```python
from build123d import *

# Parameters (mm, degrees)
SKETCH_1_W                   = 45
SKETCH_1_H                   = 15
SKETCH_1_R                   = 1.55
EXTRUDE_1_DEPTH              = 2
FILLET_1_R                   = 3
HOLE_WIZARD_M3_1_D           = 3.2
HOLE_WIZARD_M3_1_DEPTH       = 7.5
HOLE_WIZARD_M3_1_CSINK_D     = 6.6
HOLE_WIZARD_M3_1_CSINK_ANGLE = 90
HOLE_WIZARD_M3_1_TIP         = 0.96137699


with BuildPart() as part:
    # 草图1 → 凸台-拉伸1 (new body)
    with BuildSketch(Plane(origin=(0, 0, 0), x_dir=(1, 0, 0), z_dir=(0, 1, 0))):
        Rectangle(SKETCH_1_W, SKETCH_1_H)
        with Locations(Location((-19, 0, 0), (0, 0, 270))):
            Circle(SKETCH_1_R, mode=Mode.SUBTRACT)
        with BuildLine():
            ThreePointArc((-9.05, 1.675), (-9.6, 2.225), (-9.05, 2.775))
            Line((-9.05, 2.775), (-7, 2.775))
            ThreePointArc((-7, 2.775), (-6.61109127, 2.61390873), (-6.45, 2.225))
            ThreePointArc((-6.45, 2.225), (-6.61109127, 1.83609127), (-7, 1.675))
            Line((-7, 1.675), (-7, -1.675))
            ThreePointArc((-7, -1.675), (-6.61109127, -1.83609127), (-6.45, -2.225))
            ThreePointArc((-6.45, -2.225), (-6.61109127, -2.61390873), (-7, -2.775))
            Line((-7, -2.775), (-9.05, -2.775))
            ThreePointArc((-9.05, -2.775), (-9.6, -2.225), (-9.05, -1.675))
            Line((-9.05, -1.675), (-9.05, 1.675))
        make_face(mode=Mode.SUBTRACT)
        with Locations(Location((2.025, 0, 0), (0, 0, 270))):
            Circle(SKETCH_1_R, mode=Mode.SUBTRACT)
        with BuildLine():
            ThreePointArc((7, 1.675), (6.45, 2.225), (7, 2.775))
            Line((7, 2.775), (9.05, 2.775))
            ThreePointArc((9.05, 2.775), (9.43890873, 2.61390873), (9.6, 2.225))
            ThreePointArc((9.6, 2.225), (9.43890873, 1.83609127), (9.05, 1.675))
            Line((9.05, 1.675), (9.05, -1.675))
            ThreePointArc((9.05, -1.675), (9.43890873, -1.83609127), (9.6, -2.225))
            ThreePointArc((9.6, -2.225), (9.43890873, -2.61390873), (9.05, -2.775))
            Line((9.05, -2.775), (7, -2.775))
            ThreePointArc((7, -2.775), (6.45, -2.225), (7, -1.675))
            Line((7, -1.675), (7, 1.675))
        make_face(mode=Mode.SUBTRACT)
        with Locations(Location((19, 0, 0), (0, 0, 270))):
            Circle(SKETCH_1_R, mode=Mode.SUBTRACT)
    extrude(amount=EXTRUDE_1_DEPTH)

    # 圆角1
    fillet_1_edges = [part.edges().sort_by_distance(p)[0] for p in [
        (22.5, 1, 7.5),
        (-22.5, 1, 7.5),
        (-22.5, 1, -7.5),
        (22.5, 1, -7.5),
    ]]
    fillet(fillet_1_edges, radius=FILLET_1_R)

    # M3 十字槽半沉头木螺钉的锥形沉头孔1
    with Locations(Plane(origin=(0, 2, 0), x_dir=(1, 0, 0), z_dir=(0, 1, 0))):
        with Locations((2.025, 0)):
            CounterSinkHole(HOLE_WIZARD_M3_1_D / 2, HOLE_WIZARD_M3_1_CSINK_D / 2, depth=HOLE_WIZARD_M3_1_DEPTH, counter_sink_angle=HOLE_WIZARD_M3_1_CSINK_ANGLE)
            with Locations((0, 0, -(HOLE_WIZARD_M3_1_DEPTH + HOLE_WIZARD_M3_1_TIP / 2))):  # 118° drill point
                Cone(0, HOLE_WIZARD_M3_1_D / 2, HOLE_WIZARD_M3_1_TIP, mode=Mode.SUBTRACT)


solid = part.part
```
For this review, take the finished solid that the model builds, in its own axes (mm). A direction names the side the tool comes from. Coordinates: 2 decimals unless noted, no trailing zeros. Loops run counter-clockwise (first coordinate to the right, second up) from the corner with the lowest first, then second, coordinate; pieces in that order, holes last.
1. Add section A-A, the plane x = 19. Give the boundary of the cut face in (y, z).
2. Mouldability with a two-part tool opening along Z and no side actions: class faces 3 (the flat face through (-22.5, 1, 0)), 4 (the cylindrical face through (0.5, 0.15, -0.48)), 5 (the cylindrical face through (-21.64, 1.01, -6.6)), 6 (the cylindrical face through (21.6, 1.01, 6.64)) as +Z half, -Z half, draft (parallel to the pull), parting line (faces both ways), or undercut.
3. Add section B-B, the plane z = 0. Give the boundary of the cut face in (x, y) (3 decimals), then the cut area to 3 significant figures.
4. Add section C-C, the plane y = 1.1. Give the boundary of the cut face in (x, z) (3 decimals).
5. For line 1 (X direction, y = 0.7, z = 0.5); line 2 (X direction, y = 0.85, z = 2.5); line 3 (Z direction, x = 2, y = 1.85), list the stretches that pass through material, from the lowest coordinate up.
6. For faces 1 (the flat face through (22.5, 1, 0)), 2 (the flat face through (7, 1, 0)), list the 3-axis set-ups (+Z, -Z, +X, -X, +Y, -Y) from which the entire face can be reached by the end or side of a thin tool; tool diameter is ignored.
Result:
1. outline: (0, -7.5) - (2, -7.5) - (2, -1.55) - (0, -1.55) - close; (0, 1.55) - (2, 1.55) - (2, 7.5) - (0, 7.5) - close
2. face 3: draft
2. face 4: undercut
2. face 5: -Z half
2. face 6: +Z half
3. outline: (-22.5, 0) - (-20.55, 0) - (-20.55, 2) - (-22.5, 2) - close; (-17.45, 0) - (-9.05, 0) - (-9.05, 2) - (-17.45, 2) - close; (-7, 0) - (0.425, 0) - (0.425, 0.3) - (-1.275, 2) - (-7, 2) - close; (3.625, 0) - (7, 0) - (7, 2) - (5.325, 2) - (3.625, 0.3) - close; (9.05, 0) - (17.45, 0) - (17.45, 2) - (9.05, 2) - close; (20.55, 0) - (22.5, 0) - (22.5, 2) - (20.55, 2) - close
3. area: 60.1 mm2
4. outline: (-22.5, -4.5) arc R3 ccw to (-19.5, -7.5) - (19.5, -7.5) arc R3 ccw to (22.5, -4.5) - (22.5, 4.5) arc R3 ccw to (19.5, 7.5) - (-19.5, 7.5) arc R3 ccw to (-22.5, 4.5) - close; hole circle Ø3.1 at (-19, 0); hole (-9.05, -2.775) - (-7, -2.775) arc R0.55 ccw to (-7, -1.675) - (-7, 1.675) arc R0.55 ccw to (-7, 2.775) - (-9.05, 2.775) arc R0.55 ccw to (-9.05, 1.675) - (-9.05, -1.675) arc R0.55 ccw to start; hole circle Ø4.8 at (2.025, 0); hole (7, -2.775) - (9.05, -2.775) arc R0.55 ccw to (9.05, -1.675) - (9.05, 1.675) arc R0.55 ccw to (9.05, 2.775) - (7, 2.775) arc R0.55 ccw to (7, 1.675) - (7, -1.675) arc R0.55 ccw to start; hole circle Ø3.1 at (19, 0)
5. line 1: x = -22.5 to -20.47, -17.53 to -9.05, -7 to 0.09, 3.96 to 7, 9.05 to 17.53, 20.47 to 22.5
5. line 2: x = -22.5 to -9.53, -6.52 to 6.52, 9.53 to 22.5
5. line 3: z = -7.5 to -3.15, 3.15 to 7.5
6. face 1: +Z, -Z, +X, +Y, -Y
6. face 2: +Y, -Y
